from build123d import *

# Parameters (mm, degrees)
HEX_PROFILE_R                      = 25
HEX_NUT_BODY_DEPTH                 = 60
CASTELLATION_SLOT_10_WIDE_DEPTH    = 25
CASTELLATION_SLOT_PATTERN_6X_COUNT = 6


with BuildPart() as part:
    # Hex Profile → Hex Nut Body (new body)
    with BuildSketch(Plane(origin=(0, 0, 0), x_dir=(1, 0, 0), z_dir=(0, 1, 0))):
        Polygon((60.044427996, 0), (30.022213998, 52), (-30.022213998, 52), (-60.044427996, 0), (-30.022213998, -52), (30.022213998, -52), align=None)
        with Locations(Location((0, 0, 0), (0, 0, 270))):
            Circle(HEX_PROFILE_R, mode=Mode.SUBTRACT)
    extrude(amount=-HEX_NUT_BODY_DEPTH)

    # Top Chamfer Profile → Top Chamfer 10x10 (revolve, cut)
    with BuildSketch(Plane.XY, mode=Mode.PRIVATE) as top_chamfer_10x10_sk:
        Polygon((50.044427996, 0), (60.044427996, -10), (60.044427996, 0), align=None)
    revolve(top_chamfer_10x10_sk.sketch.rotate(Axis((0, -60, 0), (0, 1, 0)), 90), axis=Axis((0, -60, 0), (0, 1, 0)), mode=Mode.SUBTRACT)

    # Castellation Slot Profile → Castellation Slot 10 Wide (cut)
    with BuildSketch(Plane(origin=(0, 0, 0), x_dir=(1, 0, 0), z_dir=(0, 1, 0))):
        with BuildLine():
            Line((-5, 24.494897428), (-5, 52))
            Line((-5, 52), (5, 52))
            Line((5, 52), (5, 24.494897428))
            ThreePointArc((5, 24.494897428), (0, 25), (-5, 24.494897428))
        make_face()
    castellation_slot_10_wide = extrude(amount=-CASTELLATION_SLOT_10_WIDE_DEPTH, mode=Mode.SUBTRACT)

    # Castellation Slot Pattern 6x: Castellation Slot 10 Wide ×6 about axis
    castellation_slot_pattern_6x_axis = Axis((0, 0, 0), (0, 1, 0))
    for i in range(1, CASTELLATION_SLOT_PATTERN_6X_COUNT):
        add(castellation_slot_10_wide.rotate(castellation_slot_pattern_6x_axis, i * 360 / CASTELLATION_SLOT_PATTERN_6X_COUNT), mode=Mode.SUBTRACT)


solid = part.part
Could you check a few things on this model? Use its own coordinates, in mm. A direction names the side the tool comes from. Coordinates: 2 decimals unless noted, no trailing zeros. Order: outer loops, then holes, each group sorted by start corner. A loop starts at its lowest first (then second) coordinate and runs counter-clockwise, first axis right, second up. Notation, with made-up numbers: (10.5, 5.25) - (62.5, 5.25) arc R36 cw to (62.5, 39.25) - close; hole circle Ø6 at (-40, 65.25). An arc over 180 degrees is marked (long way). Answer in a Markdown table with one row per item. Add a question column.
(1) Will these pins go through, and if not, where does the flat tip stop? pin 1 (3 mm diameter, centred on x = -1, z = -43, fed in from +Y); pin 2 (20 mm diameter, centred on y = -8.5, z = 44.5, fed in from +X); pin 3 (12.5 mm diameter, centred on y = -14, z = 38.5, fed in from -X).
(2) If we section it at B-B, the plane x = 0: Please give me the cut outline in (y, z), then the cut area to 3 significant figures.
(3) If we section it at C-C, the plane y = -55.5: Please give me the cut outline in (x, z).
(4) If we section it at A-A, the plane y = -19: State how many separate pieces and enclosed holes the cut face has, then the cut area to 3 significant figures.
(5) If we mould it in two halves opening along Z, with no side actions, what happens to faces 4 (the face through (-30.79, -12.32, -23.55)), 5 (the face through (40, 0, 0)), 6 (the face through (0, -31, -52))? For each: released by +Z, released by -Z, zero draft, split by the parting line, or undercut.
(6) On a 3-axis mill with a long thin cutter (end or side, diameter ignored), from which of +Z, -Z, +X, -X, +Y, -Y can I reach the whole of each face in a straight line? I mean faces 1 (the face through (5, -12, -38)), 2 (the face through (33, -25, 19)), 3 (the face through (26.7, -2.8, -45.6)). Say none if no direction works.
(7) I need wall thicknesses on L1, parallel to X at y = -29, z = 0; L2, parallel to Z at x = 0, y = -38; L3, parallel to Y at x = -43.5, z = -22.5. Which ranges of each line are inside material? Lowest first, please.
Results are:
| question | item | result |
|---|---|---|
| 1 | pin 1 | stops at y = -25 |
| 1 | pin 2 | stops at x = 40.13 |
| 1 | pin 3 | stops at x = -41.42 |
| 2 | outline | (-60, -52) - (-25, -52) - (-25, -25) - (-60, -25) - close; (-60, 25) - (-25, 25) - (-25, 52) - (-60, 52) - close |
| 2 | area | 1,890 mm2 |
| 3 | outline | (-60.04, 0) - (-30.02, -52) - (30.02, -52) - (60.04, 0) - (30.02, 52) - (-30.02, 52) - close; hole circle Ø50 at (0, 0) |
| 4 | separate pieces | 6 |
| 4 | enclosed holes | 0 |
| 4 | area | 5,770 mm2 |
| 5 | face 4 | undercut |
| 5 | face 5 | zero draft |
| 5 | face 6 | released by -Z |
| 6 | face 1 | +Z, -Z, +Y |
| 6 | face 2 | +Y |
| 6 | face 3 | -Z, +X, +Y |
| 7 | L1 | x = -60.04 to -25, 25 to 60.04 |
| 7 | L2 | z = -52 to -25, 25 to 52 |
| 7 | L3 | y = -60 to -25 |
